```python
from build123d import *

# Parameters (mm, degrees)
BOSS_EXTRUDE1_DEPTH        = 5.5
SKETCH2_R                  = 8.7
BOSS_EXTRUDE2_DEPTH        = 236
BOSS_EXTRUDE3_DEPTH        = 9.5
SKETCH4_W                  = 8
SKETCH4_H                  = 5
M3_5_CLEARANCE_HOLE1_D     = 4.134
M3_5_CLEARANCE_HOLE1_DEPTH = 5.5
M3_5_CLEARANCE_HOLE1_TIP   = 1.193383006
CHAMFER1_SIZE              = 0.5415
CHAMFER2_SIZE              = 0.433


with BuildPart() as part:
    # Sketch1 → Boss-Extrude1 (new body)
    with BuildSketch(Plane(origin=(0, 0, 0), x_dir=(0, -1, 0), z_dir=(-1, 0, 0))):
        with BuildLine():
            Line((4.034538387, 9.15), (-4.034538387, 9.15))
            ThreePointArc((-4.034538387, 9.15), (-7.071067812, 7.071067812), (-9.15, 4.034538387))
            Line((-9.15, 4.034538387), (-9.15, -4.034538387))
            ThreePointArc((-9.15, -4.034538387), (-7.071067812, -7.071067812), (-4.034538387, -9.15))
            Line((-4.034538387, -9.15), (4.034538387, -9.15))
            ThreePointArc((4.034538387, -9.15), (7.071067812, -7.071067812), (9.15, -4.034538387))
            Line((9.15, -4.034538387), (9.15, 4.034538387))
            ThreePointArc((9.15, 4.034538387), (7.071067812, 7.071067812), (4.034538387, 9.15))
        make_face()
    extrude(amount=-BOSS_EXTRUDE1_DEPTH)

    # Sketch2 → Boss-Extrude2 (add)
    with BuildSketch(Plane(origin=(5.5, 0, 0), x_dir=(0, 0, -1), z_dir=(1, 0, 0))):
        with Locations(Location((0, 0, 0), (0, 0, 180))):
            Circle(SKETCH2_R)
    extrude(amount=BOSS_EXTRUDE2_DEPTH)

    # Sketch3 → Boss-Extrude3 (add)
    with BuildSketch(Plane(origin=(241.5, 0, 0), x_dir=(0, -1, 0), z_dir=(-1, 0, 0))):
        with BuildLine():
            Line((-9.15, 4.034538387), (-9.15, -4.034538387))
            ThreePointArc((-9.15, -4.034538387), (-7.071067812, -7.071067812), (-4.034538387, -9.15))
            Line((-4.034538387, -9.15), (4.034538387, -9.15))
            ThreePointArc((4.034538387, -9.15), (7.071067812, -7.071067812), (9.15, -4.034538387))
            Line((9.15, -4.034538387), (9.15, 4.034538387))
            ThreePointArc((9.15, 4.034538387), (7.071067812, 7.071067812), (4.034538387, 9.15))
            Line((4.034538387, 9.15), (-4.034538387, 9.15))
            ThreePointArc((-4.034538387, 9.15), (-7.071067812, 7.071067812), (-9.15, 4.034538387))
        make_face()
    extrude(amount=-BOSS_EXTRUDE3_DEPTH)

    # Sketch4 → Revolve1 (revolve)
    with BuildSketch(Plane.XY, mode=Mode.PRIVATE) as revolve1_sk:
        with Locations((-4, 2.5)):
            Rectangle(SKETCH4_W, SKETCH4_H)
    revolve(revolve1_sk.sketch.rotate(Axis((-8, 0, 0), (1, 0, 0)), 270), axis=Axis((-8, 0, 0), (1, 0, 0)))

    # M3.5 Clearance Hole1
    with Locations(Plane(origin=(0, 9.15, 0), x_dir=(1, 0, 0), z_dir=(0, 1, 0))):
        with Locations((246, 0)):
            Hole(M3_5_CLEARANCE_HOLE1_D / 2, depth=M3_5_CLEARANCE_HOLE1_DEPTH)
            with Locations((0, 0, -(M3_5_CLEARANCE_HOLE1_DEPTH + M3_5_CLEARANCE_HOLE1_TIP / 2))):  # 120° drill point
                Cone(0, M3_5_CLEARANCE_HOLE1_D / 2, M3_5_CLEARANCE_HOLE1_TIP, mode=Mode.SUBTRACT)

    # Sketch7 → CBORE for M13 SHSS1 (revolve, cut)
    with BuildSketch(Plane(origin=(-8, 0, 0), x_dir=(0, 0, 1), z_dir=(0, 1, 0))):
        Polygon((0, 0), (0, 143.5), (8, 143.5), (8, 13.5), (2.5, 13.5), (2.5, 0), align=None)
    revolve(axis=Axis((-14.35, 0, 0), (1, 0, 0)), mode=Mode.SUBTRACT)

    # Chamfer1
    chamfer1_edges = [part.edges().sort_by_distance(p)[0] for p in [
        (-8, 0, 5),
    ]]
    chamfer(chamfer1_edges, length=CHAMFER1_SIZE)

    # Chamfer2
    chamfer2_edges = [part.edges().sort_by_distance(p)[0] for p in [
        (248.067, 9.15, 0),
    ]]
    chamfer(chamfer2_edges, length=CHAMFER2_SIZE)


solid = part.part
```
Verification items for the finished model (mm, model axes). A direction names the side the tool comes from. Coordinates: 2 decimals unless noted, no trailing zeros. Loops run counter-clockwise (first coordinate to the right, second up) from the corner with the lowest first, then second, coordinate; pieces in that order, holes last. Notation, with made-up numbers: (-39, 9) -> (-32, 9) arc R22 ccw to (-32, 46) -> close; hole circle Ø4 at (84, -11). An arc over 180 degrees is marked (long way). Answer in a Markdown table with one row per item.
1) Depth check by flat-ended pin: P1, Ø8, axis at x = 166, y = 2.5, coming from the +Z side; P2, Ø1.5, axis at x = 224.5, y = 5, coming from the +Z side; P3, Ø6, axis at x = 22, z = 2.5, coming from the -Y side. Enter the tip coordinate at first touch or a pass-through.
The answers:
| item | result |
|---|---|
| P1 | stops at z = 8.7 |
| P2 | stops at z = 7.59 |
| P3 | stops at y = -8.7 |
2) Section check A-A (x = 99.5). Record the cut outline in (y, z).
The answers:
| item | result |
|---|---|
| outline | circle Ø17.4 at (0, 0); hole circle Ø16 at (0, 0) |
3) Draft check along X on faces 5 (the face through (2.71, 7.03, 7.11)), 6 (the face through (245.641, 2.664, -0.016)), 7 (the face through (251, 0, 0)). Enter one of: released by +X, released by -X, zero draft, split by the parting line, or undercut.
The answers:
| item | result |
|---|---|
| face 5 | zero draft |
| face 6 | undercut |
| face 7 | released by +X |
4) Access from +Z, -Z, +X, -X, +Y, -Y to the whole of each face (thin tool, end or side, straight path). Record for faces 1 (the face through (69.59, 7.81, -1.73)), 2 (the face through (248.065, 6.148, -0.091)), 3 (the face through (-1.34, 2.44, -0.54)), 4 (the face through (246.18, 7.11, -7.03)).
The answers:
| item | result |
|---|---|
| face 1 | none |
| face 2 | +Y |
| face 3 | -X |
| face 4 | -Z, +X, -X, +Y |
5) Section check B-B (y = 0). Record the cut outline in (x, z), and give its area (3 significant figures).
The answers:
| item | result |
|---|---|
| outline | (-8, -4.46) -> (-7.46, -5) -> (0, -5) -> (0, -9.15) -> (5.5, -9.15) -> (5.5, -8.7) -> (241.5, -8.7) -> (241.5, -9.15) -> (251, -9.15) -> (251, 9.15) -> (241.5, 9.15) -> (241.5, 8.7) -> (5.5, 8.7) -> (5.5, 9.15) -> (0, 9.15) -> (0, 5) -> (-7.46, 5) -> (-8, 4.46) -> (-8, 2.5) -> (5.5, 2.5) -> (5.5, 8) -> (135.5, 8) -> (135.5, -8) -> (5.5, -8) -> (5.5, -2.5) -> (-8, -2.5) -> close |
| area | 2,310 mm2 |
6) Scan lines: line 1 along X through (y, z) = (6.5, 0); line 2 along X through (y, z) = (0, -7); line 3 along Y through (x, z) = (105, 0). Record each from-to range of solid material in increasing order. Write a range as from..to.
The answers:
| item | result |
|---|---|
| line 1 | x = 0..5.5, 135.5..243.93, 248.07..251 |
| line 2 | x = 0..5.5, 135.5..251 |
| line 3 | y = -8.7..-8, 8..8.7 |
7) Section check C-C (x = 179.5). Record the cut outline in (y, z).
The answers:
| item | result |
|---|---|
| outline | circle Ø17.4 at (0, 0) |
